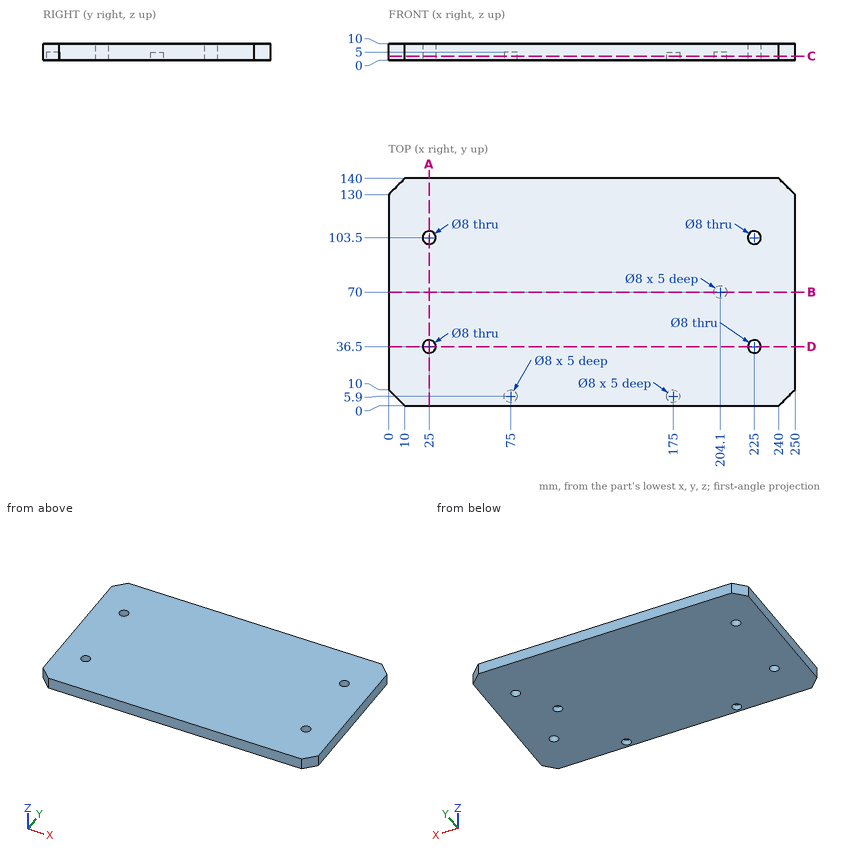
The drawing under review shows one solid part. Ordinate dimensions are in mm from its lowest x, y, z. Coordinates: 2 decimals unless noted, no trailing zeros. Order: outer loops, then holes, each group sorted by start corner. A loop starts at its lowest first (then second) coordinate and runs counter-clockwise, first axis right, second up. Notation, with made-up numbers: (55, -29) -> (91, -29) arc R19 cw to (91, 2) -> close; hole circle Ø5 at (-25.5, -19). An arc over 180 degrees is marked (long way). Answer in a Markdown table with one row per item. Add a question column.
Item 1: Clearance check with flat-ended pins moving along their axes: pin 1 (10.5 mm diameter, centred on x = 225, y = 36.5, fed in from +Z); pin 2 (7 mm diameter, centred on x = 25, y = 103.5, fed in from +Z); pin 3 (2.5 mm diameter, centred on x = 73.5, y = 7, fed in from -Z). State where each tip first meets the part, or that it passes through.
Item 2: We need section A-A on x = 25. Write out the cut boundary in (y, z), plus the area to 3 significant figures.
Item 3: We need section D-D on y = 36.5. Write out the cut boundary in (x, z), plus the area to 3 significant figures.
Item 4: To check wall thickness, follow probe 1 along Y at (x, z) = (25, 6); probe 2 along Y at (x, z) = (75, 2.9); probe 3 along Y at (x, z) = (204.1, 2.3). State the ranges of each line that lie inside material, in increasing order.
Item 5: We need section B-B on y = 70. Write out the cut boundary in (x, z), plus the area to 3 significant figures.
Item 6: We need section C-C on z = 2.5. Write out the cut boundary in (x, y), plus the area to 3 significant figures.
Final values:
| question | item | result |
|---|---|---|
| 1 | pin 1 | stops at z = 10 |
| 1 | pin 2 | passes through |
| 1 | pin 3 | stops at z = 5 |
| 2 | outline | (0, 0) -> (32.5, 0) -> (32.5, 10) -> (0, 10) -> close; (40.5, 0) -> (99.5, 0) -> (99.5, 10) -> (40.5, 10) -> close; (107.5, 0) -> (140, 0) -> (140, 10) -> (107.5, 10) -> close |
| 2 | area | 1,240 mm2 |
| 3 | outline | (0, 0) -> (21, 0) -> (21, 10) -> (0, 10) -> close; (29, 0) -> (221, 0) -> (221, 10) -> (29, 10) -> close; (229, 0) -> (250, 0) -> (250, 10) -> (229, 10) -> close |
| 3 | area | 2,340 mm2 |
| 4 | probe 1 | y = 0 to 32.5, 40.5 to 99.5, 107.5 to 140 |
| 4 | probe 2 | y = 0 to 1.9, 9.9 to 140 |
| 4 | probe 3 | y = 0 to 66, 74 to 140 |
| 5 | outline | (0, 0) -> (200.1, 0) -> (200.1, 5) -> (208.1, 5) -> (208.1, 0) -> (250, 0) -> (250, 10) -> (0, 10) -> close |
| 5 | area | 2,460 mm2 |
| 6 | outline | (0, 10) -> (10, 0) -> (240, 0) -> (250, 10) -> (250, 130) -> (240, 140) -> (10, 140) -> (0, 130) -> close; hole circle Ø8 at (25, 36.5); hole circle Ø8 at (25, 103.5); hole circle Ø8 at (75, 5.9); hole circle Ø8 at (175, 5.9); hole circle Ø8 at (204.1, 70); hole circle Ø8 at (225, 36.5); hole circle Ø8 at (225, 103.5) |
| 6 | area | 34,400 mm2 |
